```python
from build123d import *

# Parameters (mm, degrees)
SKETCH5_R          = 1.5
CUT_EXTRUDE4_DEPTH = 164


with BuildPart() as part:
    # Sketch4 → Revolve2 (revolve)
    with BuildSketch(Plane(origin=(0, 0, 0), x_dir=(0, 0, -1), z_dir=(1, 0, 0))):
        Polygon((-80, 0), (-80, 12.5), (-77, 12.5), (-77, 7.5), (-70, 7.5), (-70, 3), (0, 3), (0, 0), align=None)
    revolve2 = revolve(axis=Axis((0, 0, 0), (0, 0, 1)))

    # Mirror1: Revolve2 across plane
    add(revolve2.mirror(Plane(origin=(0, 0, 0), x_dir=(1, 0, 0), z_dir=(0, 0, -1))))

    # Sketch5 → Cut-Extrude4 (cut)
    with BuildSketch(Plane(origin=(0, 0, -80), x_dir=(-1, 0, 0), z_dir=(0, 0, -1))):
        with Locations(Location((10, 0, 0), (0, 0, 90))):
            Circle(SKETCH5_R)
        with Locations(Location((0, -10, 0), (0, 0, 90))):
            Circle(SKETCH5_R)
        with Locations(Location((-10, 0, 0), (0, 0, 90))):
            Circle(SKETCH5_R)
        with Locations(Location((0, 10, 0), (0, 0, 90))):
            Circle(SKETCH5_R)
    extrude(amount=-CUT_EXTRUDE4_DEPTH, mode=Mode.SUBTRACT)


solid = part.part
```
Read the model definition and answer for the solid it produces. Units are mm, in the model's axes. A direction names the side the tool comes from. Round coordinates to 2 decimals unless told otherwise and drop trailing zeros. Write each loop counter-clockwise with the first axis right and the second up, starting at its lowest first coordinate (ties: lowest second). Pieces come first, ordered by that corner, then holes. Notation, with made-up numbers: (19, -19.75) - (33, -19.75) arc R22 cw to (33, -1.75) - close; hole circle Ø9 at (-9.75, 87). An arc over 180 degrees is marked (long way). Use CSV: the item, a comma, the result in double quotes.
Q1. A tool of negligible diameter and unlimited length cuts with its end or side. For faces 1 (the flat face through (0, 0, -80)), 2 (the flat face through (8, 0, 77)), from which of +Z, -Z, +X, -X, +Y, -Y can it reach the whole face along a straight path? Write none if from no direction.
Values:
face 1,"-Z, +X, -X, +Y, -Y"
face 2,"none"
Q2. Straight lines are drawn through the part: line 1 along X through (y, z) = (0, -79.1); line 2 along X through (y, z) = (-10, 78.4); line 3 along Z through (x, y) = (-7.5, -9). For each, find the intervals that lie inside material, in ascending order.
Values:
line 1,"x = -12.5 to -11.5, -8.5 to 8.5, 11.5 to 12.5"
line 2,"x = -7.5 to -1.5, 1.5 to 7.5"
line 3,"z = -80 to -77, 77 to 80"
Q3. Find section A-A, the plane x = -10. Write down the section's boundary in (y, z).
Values:
outline,"(-7.5, -80) - (-1.5, -80) - (-1.5, -77) - (-7.5, -77) - close; (-7.5, 77) - (-1.5, 77) - (-1.5, 80) - (-7.5, 80) - close; (1.5, -80) - (7.5, -80) - (7.5, -77) - (1.5, -77) - close; (1.5, 77) - (7.5, 77) - (7.5, 80) - (1.5, 80) - close"
Q4. Determine the mould class of faces 3 (the flat face through (0, 0, 80)), 4 (the cylindrical face through (-3.755, 11.923, -78.479)), 5 (the flat face through (8, 0, -77)) for opening direction Z: +Z half, -Z half, draft (parallel to the pull), parting line (faces both ways), or undercut.
Values:
face 3,"+Z half"
face 4,"draft"
face 5,"undercut"
Q5. Find section C-C, the plane x = 0. Count the separate pieces of the cut face and the enclosed holes in it, then the cut area to 3 significant figures.
Values:
separate pieces,"5"
enclosed holes,"0"
area,"1,160 mm²"
Q6. Each of these flat-tipped pins is pushed along its axis until it touches: pin 1 Ø10 at (y, z) = (-7.5, 25) entering from +X; pin 2 Ø2.5 at (x, y) = (10, 0) entering from -Z; pin 3 Ø10 at (y, z) = (-1.5, 6.5) entering from -X; pin 4 Ø12 at (x, z) = (3.5, 16.5) entering from +Y. Where does it stop, or does it pass through?
Values:
pin 1,"stops at x = 1.66"
pin 2,"passes through"
pin 3,"stops at x = -3"
pin 4,"stops at y = 3"
